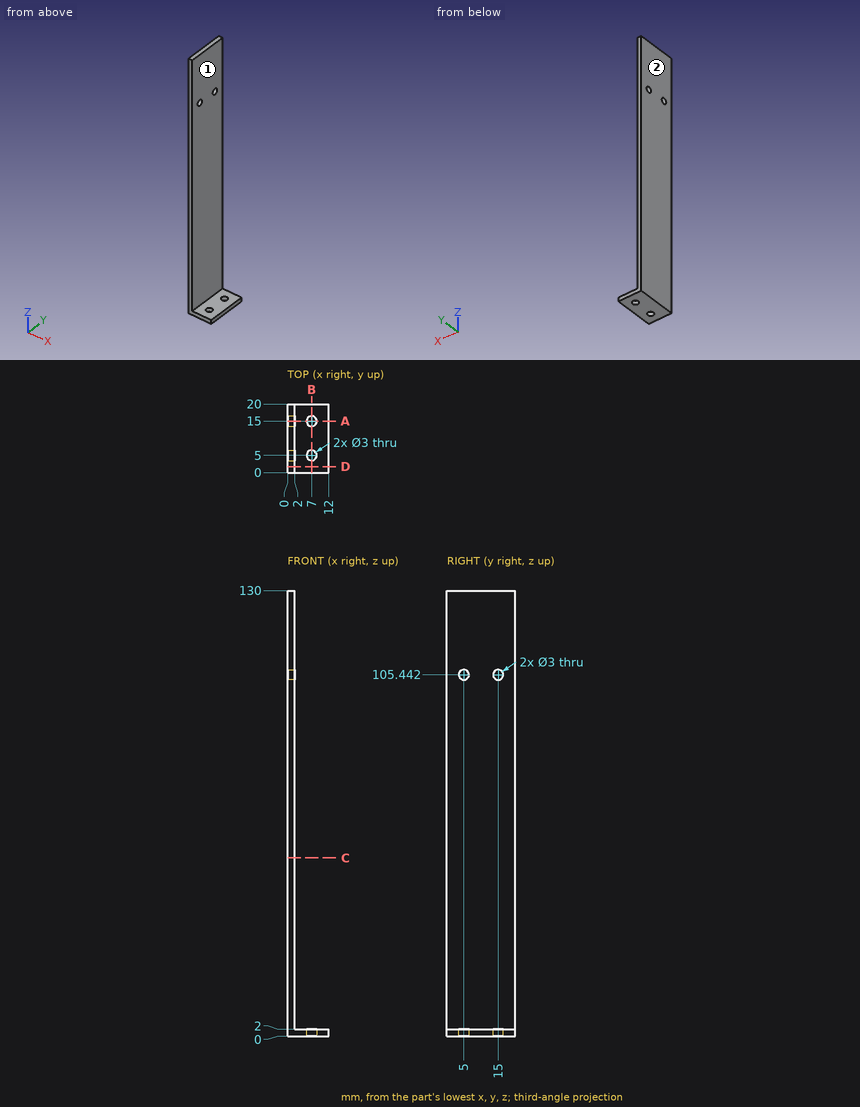
Check sheet for the drawn part. Datum: minimum x, y, z corner. Units: mm. A direction names the side the tool comes from. Give positions to 0.01 mm unless a question says otherwise; leave off trailing zeros. Order: outer loops, then holes, each group sorted by start corner. A loop starts at its lowest first (then second) coordinate and runs counter-clockwise, first axis right, second up.
1. Sectioned sample at C-C (z = 52). Record the boundary of the cut face in (x, y).
Completed:
outline: (0, 0) - (2, 0) - (2, 20) - (0, 20) - close
2. Sectioned sample at B-B (x = 7). Record the boundary of the cut face in (y, z).
Completed:
outline: (0, 0) - (3.5, 0) - (3.5, 2) - (0, 2) - close; (6.5, 0) - (13.5, 0) - (13.5, 2) - (6.5, 2) - close; (16.5, 0) - (20, 0) - (20, 2) - (16.5, 2) - close
3. Sectioned sample at D-D (y = 1.75). Record the boundary of the cut face in (x, z), then the cut area to 3 significant figures.
Completed:
outline: (0, 0) - (12, 0) - (12, 2) - (2, 2) - (2, 130) - (0, 130) - close
area: 280 mm2
4. Depth check by flat-ended pin: pin 1 (3 mm diameter, centred on x = 8.5, y = 8.5, fed in from +Z); pin 2 (2.5 mm diameter, centred on x = 7, y = 15, fed in from +Z); pin 3 (5 mm diameter, centred on y = 5, z = 105.44, fed in from +X). Enter the tip coordinate at first touch or a pass-through.
Completed:
pin 1: stops at z = 2
pin 2: passes through
pin 3: stops at x = 2
5. Scan lines: line 1 (Y direction, x = 7, z = 1.35); line 2 (X direction, y = 4.25, z = 60). Record each from-to range of solid material in increasing order.
Completed:
line 1: y = 0 to 3.5, 6.5 to 13.5, 16.5 to 20
line 2: x = 0 to 2
6. Sectioned sample at A-A (y = 15). Record the boundary of the cut face in (x, z), then the cut area to 3 significant figures.
Completed:
outline: (0, 0) - (5.5, 0) - (5.5, 2) - (2, 2) - (2, 103.94) - (0, 103.94) - close; (0, 106.94) - (2, 106.94) - (2, 130) - (0, 130) - close; (8.5, 0) - (12, 0) - (12, 2) - (8.5, 2) - close
area: 268 mm2
7. Access from +Z, -Z, +X, -X, +Y, -Y to the whole of each face (thin tool, end or side, straight path). Record for the marked faces 1 and 2.
Completed:
face 1: +Z, +X, +Y, -Y
face 2: +Z, -Z, -X, +Y, -Y
